from build123d import *

# Parameters (mm, degrees)
SKETCH_1_R      = 38
EXTRUDE_1_DEPTH = 675
SKETCH_2_R      = 8
EXTRUDE_2_DEPTH = 50


with BuildPart() as part:
    # 草图1 → 凸台-拉伸1 (new, symmetric)
    with BuildSketch(Plane.XY):
        Circle(SKETCH_1_R)
    extrude(amount=EXTRUDE_1_DEPTH, both=True)

    # 草图2 → 凸台-拉伸2 (add, symmetric)
    with BuildSketch(Plane.XY.offset(675)):
        Circle(SKETCH_2_R)
    extrude_2 = extrude(amount=EXTRUDE_2_DEPTH, both=True)

    # 镜向1: 凸台-拉伸2 across plane
    add(extrude_2.mirror(Plane.XY))


solid = part.part
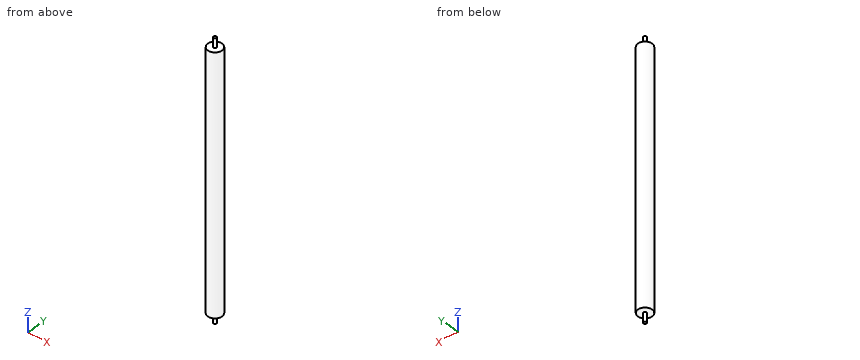
Input: part model. Units: mm. Frame: model coordinates. Round coordinates to 2 decimals unless told otherwise and drop trailing zeros. Loops run counter-clockwise (first coordinate to the right, second up) from the corner with the lowest first, then second, coordinate; pieces in that order, holes last. Notation, with made-up numbers: M 69.25,5 L 91.25,5 A33 ccw 91.25,43 Z; hole C 31.5,88.25 d8. An arc over 180 degrees is marked long. Answer as CSV lines item,"result". Start each with the question number.
(1) Line query: line 1 (Z direction, x = 16.5, y = 20); line 2 (X direction, y = 3, z = 563); line 3 (Y direction, x = 6, z = 478). Output: solid intervals per line, ascending. Write a range as [from, to].
(2) First-contact query: pin 1 (1 mm diameter, centred on x = 22, z = -166, fed in from -Y); pin 2 (1.5 mm diameter, centred on x = -11.5, y = -24.5, fed in from +Z); pin 3 (4 mm diameter, centred on x = -28, z = 145.5, fed in from -Y). Flat tips, straight axial feed; report the tip coordinate or a pass-through.
(3) Section C-C, the plane x = -20.5. Output: boundary loops of the cut face in (y, z), plus the area to 3 significant figures.
(4) Section A-A, the plane z = -43. Output: boundary loops of the cut face in (x, y), plus the area to 3 significant figures.
(5) Section B-B, the plane y = 23.5. Output: boundary loops of the cut face in (x, z).
Values found:
1,line 1,"z = [-675, 675]"
1,line 2,"x = [-37.88, 37.88]"
1,line 3,"y = [-37.52, 37.52]"
2,pin 1,"stops at y = -31.33"
2,pin 2,"stops at z = 675"
2,pin 3,"stops at y = -27.71"
3,outline,"M -32,-675 L 32,-675 L 32,675 L -32,675 Z"
3,area,"86,400 mm²"
4,outline,"C 0,0 d76"
4,area,"4,540 mm²"
5,outline,"M -29.86,-675 L 29.86,-675 L 29.86,675 L -29.86,675 Z"
